Can you work these out from the drawing? Everything is in mm from the part's minimum corner. Coordinates: 2 decimals unless noted, no trailing zeros. Write each loop counter-clockwise with the first axis right and the second up, starting at its lowest first coordinate (ties: lowest second). Pieces come first, ordered by that corner, then holes. Notation, with made-up numbers: M 8,44 L 21,44 A7 cw 21,52 Z; hole C -31,-38 d1. An arc over 180 degrees is marked long. Write item = value, one per line.
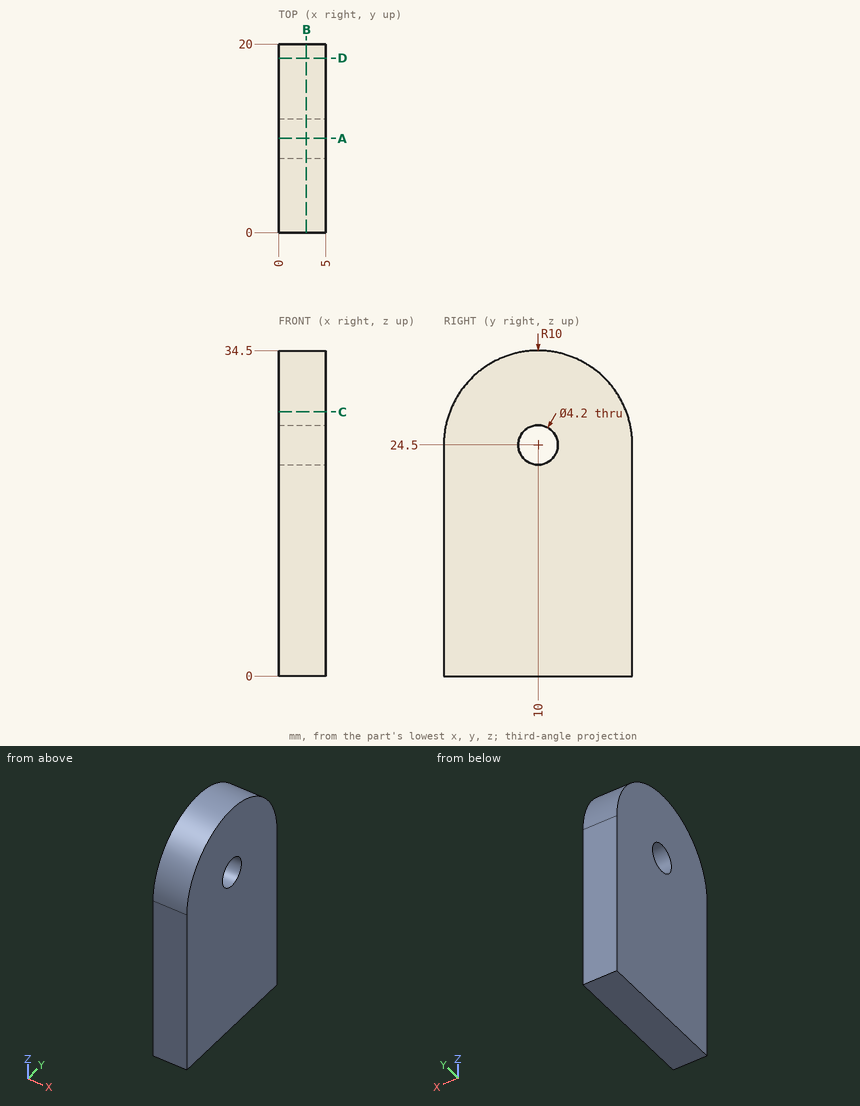
Item 1: Imagine slicing it at D-D (y = 18.5). Write out the boundary of the cut face in (x, z), and give its area (3 significant figures).
Numbers:
outline = M 0,0 L 5,0 L 5,29.77 L 0,29.77 Z
area = 149 mm²
Item 2: Imagine slicing it at A-A (y = 10). Write out the boundary of the cut face in (x, z).
Numbers:
outline = M 0,0 L 5,0 L 5,22.4 L 0,22.4 Z; M 0,26.6 L 5,26.6 L 5,34.5 L 0,34.5 Z
Item 3: Imagine slicing it at B-B (x = 2.95). Write out the boundary of the cut face in (y, z).
Numbers:
outline = M 0,0 L 20,0 L 20,24.5 A10 ccw 0,24.5 Z; hole C 10,24.5 d4.2
Item 4: If I drill on line 1 along Y through (x, z) = (3.7, 24.5); line 2 along Z through (x, y) = (3.9, 10); line 3 along Y through (x, z) = (3.9, 24), over which ranges is the centre line in solid material (lowest first)?
Numbers:
line_1 = 0 to 7.9, 12.1 to 20
line_2 = 0 to 22.4, 26.6 to 34.5
line_3 = 0 to 7.96, 12.04 to 20
Item 5: Imagine slicing it at C-C (z = 28). Write out the boundary of the cut face in (x, y), and give its area (3 significant figures).
Numbers:
outline = M 0,0.63 L 5,0.63 L 5,19.37 L 0,19.37 Z
area = 93.7 mm²
